Verification items for the finished model (mm, model axes). A direction names the side the tool comes from. Coordinates: 2 decimals unless noted, no trailing zeros. Loops run counter-clockwise (first coordinate to the right, second up) from the corner with the lowest first, then second, coordinate; pieces in that order, holes last. Notation, with made-up numbers: (41, 49.5) - (62, 49.5) arc R27 ccw to (62, 87.5) - close; hole circle Ø1 at (6, -16.75). An arc over 180 degrees is marked (long way). One line per item, written item: value. Start each with the question number.
(1) Section check C-C (z = 3.7). Record the boundary of the cut face in (x, y).
(2) Set-up check for faces 4 (the face through (-2, 8, 3)), 5 (the face through (-6, 8, 3.3)), 6 (the face through (-6, -6, 2)): record each of +Z, -Z, +X, -X, +Y, -Y from which the full face is reachable in a straight line by a thin tool's end or side.
(3) Draft check along X on faces 1 (the face through (9.64, -0.27, 2.66)), 2 (the face through (9, 8, 3)), 3 (the face through (5, -6, 3.4)). Enter one of: +X half, -X half, draft (parallel to the pull), parting line (faces both ways), or undercut.
(4) Thickness scan on probe 1 along Y at (x, z) = (10.5, 2.85); probe 2 along Y at (x, z) = (7.5, 0.9); probe 3 along X at (y, z) = (9.75, 3.2). Record the ranges inside material, lowest first. Write a range as [from, to].
(5) Section check D-D (y = 0). Record the boundary of the cut face in (x, z), plus the area to 3 significant figures.
(6) Section check A-A (y = 7.75). Record the boundary of the cut face in (x, z).
(7) Gauge pin test, flat ends, axial feed: P1, Ø7.5, axis at x = -7, y = 10, coming from the -Z side; P2, Ø2, axis at x = -6.5, y = 9, coming from the +Z side; P3, Ø1.1, axis at x = -10.5, y = 0, coming from the -Z side; P4, Ø4, axis at x = 6, y = -5.5, coming from the -Z side. Record the tip position at first contact, or that the pin passes through.
(8) Section check B-B (x = -10.5). Record the boundary of the cut face in (y, z), plus the area to 3 significant figures.
```python
from build123d import *

# Parameters (mm, degrees)
SKETCH_1_W      = 25
SKETCH_1_H      = 8
SKETCH_1_R      = 0.9
EXTRUDE_1_DEPTH = 5.4
EXTRUDE_2_DEPTH = 3.65
SKETCH_3_W      = 7
SKETCH_3_H      = 1.2
EXTRUDE_3_DEPTH = 8.75
CHAMFER_1_SIZE  = 0.3
FILLET_1_R      = 1


with BuildPart() as part:
    # 草图1 → 凸台-拉伸1 (new body)
    with BuildSketch(Plane.XY):
        Rectangle(SKETCH_1_W, SKETCH_1_H)
        with Locations(Location((10.5, 0, 0), (0, 0, 180))):
            Circle(SKETCH_1_R, mode=Mode.SUBTRACT)
        with Locations(Location((-10.5, 0, 0), (0, 0, 180))):
            Circle(SKETCH_1_R, mode=Mode.SUBTRACT)
    extrude(amount=EXTRUDE_1_DEPTH)

    # 草图2 → 凸台-拉伸2 (add)
    with BuildSketch(Plane(origin=(0, -4, 0), x_dir=(-1, 0, 0), z_dir=(0, -1, 0))):
        with BuildLine():
            Line((-3, -3.4), (-8, -3.4))
            ThreePointArc((-8, -3.4), (-8.7, -2.7), (-8, -2))
            Line((-8, -2), (-3, -2))
            ThreePointArc((-3, -2), (-2.3, -2.7), (-3, -3.4))
        make_face()
        with BuildLine():
            Line((3, -3.4), (8, -3.4))
            ThreePointArc((8, -3.4), (8.7, -2.7), (8, -2))
            Line((8, -2), (3, -2))
            ThreePointArc((3, -2), (2.3, -2.7), (3, -3.4))
        make_face()
    extrude(amount=EXTRUDE_2_DEPTH)

    # 草图3 → 凸台-拉伸3 (add)
    with BuildSketch(Plane(origin=(0, 4, 0), x_dir=(1, 0, 0), z_dir=(0, 1, 0))):
        with Locations((5.5, -2.7)):
            Rectangle(SKETCH_3_W, SKETCH_3_H)
        with Locations((-5.5, -2.7)):
            Rectangle(SKETCH_3_W, SKETCH_3_H)
    extrude(amount=EXTRUDE_3_DEPTH)

    # 倒角1
    chamfer_1_edges = [part.edges().sort_by_distance(p)[0] for p in [
        (9, 12.75, 2.7),
        (5.5, 12.75, 2.1),
        (2, 12.75, 2.7),
        (5.5, 12.75, 3.3),
        (-2, 12.75, 2.7),
        (-5.5, 12.75, 2.1),
        (-9, 12.75, 2.7),
        (-5.5, 12.75, 3.3),
    ]]
    chamfer(chamfer_1_edges, length=CHAMFER_1_SIZE)

    # 圆角1
    fillet_1_edges = [part.edges().sort_by_distance(p)[0] for p in [
        (12.5, -4, 2.7),
        (-12.5, -4, 2.7),
        (-12.5, 4, 2.7),
        (12.5, 4, 2.7),
    ]]
    fillet(fillet_1_edges, radius=FILLET_1_R)


solid = part.part
```
Responses:
1. outline: (-12.5, -3) arc R1 ccw to (-11.5, -4) - (11.5, -4) arc R1 ccw to (12.5, -3) - (12.5, 3) arc R1 ccw to (11.5, 4) - (-11.5, 4) arc R1 ccw to (-12.5, 3) - close; hole circle Ø1.8 at (-10.5, 0); hole circle Ø1.8 at (10.5, 0)
2. face 4: +Z, -Z, +Y
2. face 5: +Z, +X, -X, +Y
2. face 6: -Z, +X, -X, -Y
3. face 1: undercut
3. face 2: +X half
3. face 3: draft
4. probe 1: y = [-4, -0.9], [0.9, 4]
4. probe 2: y = [-4, 4]
4. probe 3: x = [-9, -2], [2, 9]
5. outline: (-12.5, 0) - (-11.4, 0) - (-11.4, 5.4) - (-12.5, 5.4) - close; (-9.6, 0) - (9.6, 0) - (9.6, 5.4) - (-9.6, 5.4) - close; (11.4, 0) - (12.5, 0) - (12.5, 5.4) - (11.4, 5.4) - close
5. area: 116 mm²
6. outline: (-9, 2.1) - (-2, 2.1) - (-2, 3.3) - (-9, 3.3) - close; (2, 2.1) - (9, 2.1) - (9, 3.3) - (2, 3.3) - close
7. P1: stops at z = 2.1
7. P2: stops at z = 3.3
7. P3: passes through
7. P4: stops at z = 0
8. outline: (-4, 0) - (-0.9, 0) - (-0.9, 5.4) - (-4, 5.4) - close; (0.9, 0) - (4, 0) - (4, 5.4) - (0.9, 5.4) - close
8. area: 33.5 mm²
